Design review of the part built by this model. Coordinates are the model's own, in mm. Face numbers are marked on the shaded views. Coordinates: 2 decimals unless noted, no trailing zeros. Write each loop counter-clockwise with the first axis right and the second up, starting at its lowest first coordinate (ties: lowest second). Pieces come first, ordered by that corner, then holes. Notation, with made-up numbers: M 17.5,75.5 L 27.5,75.5 A25 ccw 27.5,89.5 Z; hole C 67.5,85 d3. An arc over 180 degrees is marked long. Write item = value, one per line.
```python
from build123d import *

# Parameters (mm, degrees)
SKETCH1_W           = 12
SKETCH1_H           = 12
SKETCH1_R           = 3.674588618
BOSS_EXTRUDE1_DEPTH = 5


with BuildPart() as part:
    # Sketch1 → Boss-Extrude1 (new body)
    with BuildSketch(Plane.XY):
        with Locations((-27.065651732, 0)):
            Rectangle(SKETCH1_W, SKETCH1_H)
        with Locations((-27.065651732, 0)):
            Circle(SKETCH1_R, mode=Mode.SUBTRACT)
    extrude(amount=-BOSS_EXTRUDE1_DEPTH)


solid = part.part
```
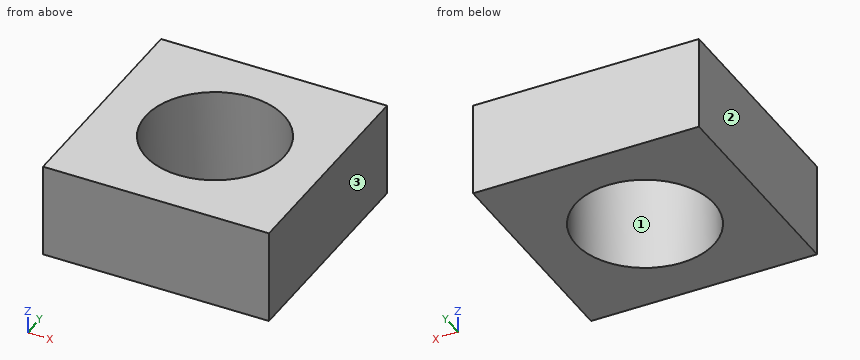
Q1. Consider section A-A, the plane y = 0. State the section outline as (x, z) points, and give its area (3 significant figures).
Check result:
outline = M -33.07,-5 L -30.74,-5 L -30.74,0 L -33.07,0 Z; M -23.39,-5 L -21.07,-5 L -21.07,0 L -23.39,0 Z
area = 23.3 mm²
Q2. The part is to be moulded in two halves that separate along X. For the marked faces 1, 2 and 3, say which applies: +X half, -X half, draft (parallel to the pull), parting line (faces both ways), or undercut.
Check result:
face_1 = undercut
face_2 = -X half
face_3 = +X half
Q3. Consider section C-C, the plane x = -24.25. State the section outline as (y, z) points.
Check result:
outline = M -6,-5 L -2.36,-5 L -2.36,0 L -6,0 Z; M 2.36,-5 L 6,-5 L 6,0 L 2.36,0 Z
Q4. Wall thickness on line 1 (Y direction, x = -27, z = -0.7); line 2 (X direction, y = -2, z = -4.4); line 3 (Y direction, x = -25.5, z = -2.75): over which ranges is each line inside the solid? List them lowest first.
Check result:
line_1 = -6 to -3.67, 3.67 to 6
line_2 = -33.07 to -30.15, -23.98 to -21.07
line_3 = -6 to -3.32, 3.32 to 6
Q5. Consider section B-B, the plane z = -4.25. State the section outline as (x, y) points, and give its area (3 significant figures).
Check result:
outline = M -33.07,-6 L -21.07,-6 L -21.07,6 L -33.07,6 Z; hole C -27.07,0 d7.35
area = 102 mm²
